Verification items for the finished model (mm, model axes). Give positions to 0.01 mm unless a question says otherwise; leave off trailing zeros. Loops run counter-clockwise (first coordinate to the right, second up) from the corner with the lowest first, then second, coordinate; pieces in that order, holes last. Notation, with made-up numbers: (61.25, 4) -> (82.25, 4) arc R18 ccw to (82.25, 13) -> close; hole circle Ø11 at (44.25, 88.5). An arc over 180 degrees is marked (long way). Use one line per item in the form item = value. Start each with the question number.
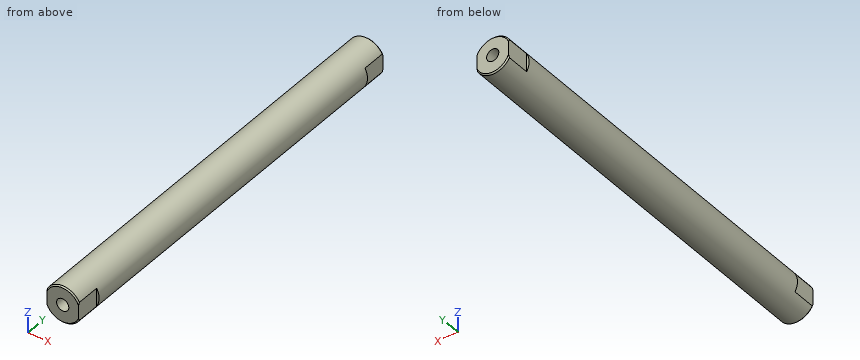
from build123d import *

# Parameters (mm, degrees)
SKETCH_1_R          = 7.5
EXTRUDE_1_DEPTH     = 84
CHAMFER_1_SIZE      = 0.5
SKETCH_4_W          = 1
SKETCH_4_H          = 10
CUT_EXTRUDE_1_DEPTH = 10


with BuildPart() as part:
    # 草图1 → 凸台-拉伸1 (new, symmetric)
    with BuildSketch(Plane(origin=(0, 0, 0), x_dir=(1, 0, 0), z_dir=(0, 1, 0))):
        with Locations(Location((0, 0, 0), (0, 0, 90))):
            Circle(SKETCH_1_R)
    extrude(amount=EXTRUDE_1_DEPTH, both=True)

    # 倒角1
    chamfer_1_edges = [part.edges().sort_by_distance(p)[0] for p in [
        (0, -84, 7.5),
        (0, 84, 7.5),
    ]]
    chamfer(chamfer_1_edges, length=CHAMFER_1_SIZE)

    # 草图2 → M6 螺纹孔1 (revolve, cut)
    with BuildSketch(Plane(origin=(0, 84, 0), x_dir=(0, 0, 1), z_dir=(1, 0, 0))):
        Polygon((0, 0), (0, 18.502151548), (2.5, 17), (2.5, 0), align=None)
    hole_wizard_m6_1 = revolve(axis=Axis((0, 90.35, 0), (0, -1, 0)), mode=Mode.SUBTRACT)

    # 镜向1: M6 螺纹孔1 across plane
    add(hole_wizard_m6_1.mirror(Plane.ZX), mode=Mode.SUBTRACT)

    # 草图4 → 切除-拉伸1 (cut, symmetric)
    with BuildSketch(Plane.XY):
        with Locations((-7, 79)):
            Rectangle(SKETCH_4_W, SKETCH_4_H)
        with Locations((7, 79)):
            Rectangle(SKETCH_4_W, SKETCH_4_H)
        with Locations((7, -79)):
            Rectangle(SKETCH_4_W, SKETCH_4_H)
        with Locations((-7, -79)):
            Rectangle(SKETCH_4_W, SKETCH_4_H)
    extrude(amount=CUT_EXTRUDE_1_DEPTH, both=True, mode=Mode.SUBTRACT)


solid = part.part
Item 1: Gauge pin test, flat ends, axial feed: pin 1 Ø3 at (y, z) = (-48.5, 3.5) entering from +X; pin 2 Ø8 at (x, y) = (2.5, 58) entering from -Z; pin 3 Ø3.5 at (y, z) = (-78.5, 0.5) entering from +X; pin 4 Ø3 at (x, z) = (0, 0) entering from -Y. Record the tip position at first contact, or that the pin passes through.
Item 2: Sectioned sample at A-A, the plane y = -27.5. Enter the section's corners in (x, z).
Item 3: Material ranges on line 1 (X direction, y = -77, z = 0); line 2 (X direction, y = 72.25, z = 0); line 3 (X direction, y = 52.5, z = 0.25), recorded low to high.
Outcome:
q1.pin_1 = 7.23
q1.pin_2 = -7.5
q1.pin_3 = 6.5
q1.pin_4 = -66.4
q2.outline = circle Ø15 at (0, 0)
q3.line_1 = -6.5 to -2.5, 2.5 to 6.5
q3.line_2 = -7.5 to -2.5, 2.5 to 7.5
q3.line_3 = -7.5 to 7.5
